from build123d import *

# Parameters (mm, degrees)
SKETCH1_R           = 5
BOSS_EXTRUDE1_DEPTH = 5


with BuildPart() as part:
    # Sketch1 → Boss-Extrude1 (new, symmetric)
    with BuildSketch(Plane.XY):
        with BuildLine():
            Line((0, 10), (30, 10))
            Line((30, 10), (30, -10))
            Line((30, -10), (0, -10))
            ThreePointArc((0, -10), (-10, 0), (0, 10))
        make_face()
        Circle(SKETCH1_R, mode=Mode.SUBTRACT)
    extrude(amount=BOSS_EXTRUDE1_DEPTH, both=True)

    # Sketch2 → Revolve1 (revolve)
    with BuildSketch(Plane.XY, mode=Mode.PRIVATE) as revolve1_sk:
        Polygon((30, 0), (30, -5), (430, -5), (430, -15), (450, -15), (450, 0), align=None)
    revolve(revolve1_sk.sketch.rotate(Axis((450, 0, 0), (-1, 0, 0)), 180), axis=Axis((450, 0, 0), (-1, 0, 0)))


solid = part.part
Here's how the part is built. I have some questions about the finished solid (model axes, mm). A direction names the side the tool comes from. Give positions to 0.01 mm unless a question says otherwise; leave off trailing zeros. Loops run counter-clockwise (first coordinate to the right, second up) from the corner with the lowest first, then second, coordinate; pieces in that order, holes last. Notation, with made-up numbers: (63.25, 52) -> (109.25, 52) arc R28 ccw to (109.25, 87) -> close; hole circle Ø5 at (50.5, -12.5). An arc over 180 degrees is marked (long way). Answer as a JSON object with one key per item and string values. Group by question number.
Item 1: Will these pins go through, and if not, where does the flat tip stop? pin 1 (6 mm diameter, centred on x = 0.5, y = 4, fed in from +Z); pin 2 (10 mm diameter, centred on x = 181.5, z = 7, fed in from -Y); pin 3 (4 mm diameter, centred on x = 55.5, y = 4, fed in from -Z).
Item 2: I need wall thicknesses on L1, parallel to Y at x = 0, z = -1; L2, parallel to X at y = 10.25, z = -7; L3, parallel to X at y = -4.5, z = 2.75. Which ranges of each line are inside material? Lowest first, please.
Item 3: Thinking about a two-plate mould opening in Y: for faces 6 (the cylindrical face through (-1.08, -4.88, -0.07)), 7 (the cylindrical face through (233, -5, 0)), 8 (the flat face through (450, 0, 0)), 9 (the flat face through (15, 10, 0)), which applies, pulls with the +Y half, pulls with the -Y half, needs draft (parallel to the pull), parting line crosses it, or undercut?
Item 4: On a 3-axis mill with a long thin cutter (end or side, diameter ignored), from which of +Z, -Z, +X, -X, +Y, -Y can I reach the whole of each face in a straight line? I mean faces 1 (the flat face through (10, 0, 5)), 2 (the flat face through (10, 0, -5)), 3 (the flat face through (430, 4, -4)), 4 (the flat face through (30, -7, 0)), 5 (the flat face through (15, -10, 0)). Say none if no direction works.
Item 5: Imagine slicing it at A-A on z = 0. Write out the boundary of the cut face in (x, y), then the cut area to 3 significant figures.
Item 6: Imagine slicing it at B-B on x = 260.5. Write out the boundary of the cut face in (y, z), then the cut area to 3 significant figures.
Answer list:
{
 "1": {"pin 1": "stops at z = 5", "pin 2": "stops at y = -4.58", "pin 3": "stops at z = -4.58"},
 "2": {"L1": "y = -10 to -5, 5 to 10", "L2": "x = 430 to 450", "L3": "x = -8.93 to -2.18, 2.18 to 30, 430 to 450"},
 "3": {"face 6": "undercut", "face 7": "parting line crosses it", "face 8": "needs draft", "face 9": "pulls with the +Y half"},
 "4": {"face 1": "+Z, -X, +Y, -Y", "face 2": "-Z, -X, +Y, -Y", "face 3": "none", "face 4": "-Y", "face 5": "+Z, -Z, -X, -Y"},
 "5": {"outline": "(0, -10) -> (30, -10) -> (30, -5) -> (430, -5) -> (430, -15) -> (450, -15) -> (450, 15) -> (430, 15) -> (430, 5) -> (30, 5) -> (30, 10) -> (0, 10) arc R10 ccw to start; hole circle Ø10 at (0, 0)", "area": "5,280 mm2"},
 "6": {"outline": "circle Ø10 at (0, 0)", "area": "78.5 mm2"}
}
